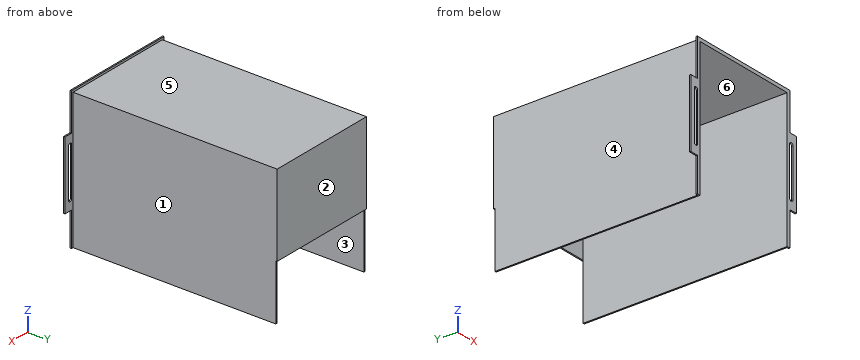
```python
from build123d import *

# Parameters (mm, degrees)
BOSS_EXTRUDE1_DEPTH     = 300
SKETCH4_W               = 15
SKETCH4_H               = 100
BOSS_EXTRUDE3_DEPTH     = 2
CUT_EXTRUDE2_DEPTH      = 402.657814564
CUT_EXTRUDE2_DEPTH_BACK = 402.657814564
SKETCH6_W               = 164
SKETCH6_H               = 120
BOSS_EXTRUDE4_DEPTH     = 2
BOSS_EXTRUDE5_DEPTH     = 2


with BuildPart() as part:
    # Sketch1 → Boss-Extrude1 (new body)
    with BuildSketch(Plane(origin=(0, 0, 0), x_dir=(1, 0, 0), z_dir=(0, 1, 0))):
        Polygon((160, 0), (160, 200), (162, 200), (162, -2), (-2, -2), (-2, 200), (0, 200), (0, 0), align=None)
    extrude(amount=BOSS_EXTRUDE1_DEPTH)

    # Sketch4 → Boss-Extrude3 (add)
    with BuildSketch(Plane.XZ):
        with Locations((-9.5, -100)):
            Rectangle(SKETCH4_W, SKETCH4_H)
        with Locations((169.5, -100)):
            Rectangle(SKETCH4_W, SKETCH4_H)
    extrude(amount=-BOSS_EXTRUDE3_DEPTH)

    # Sketch5 → Cut-Extrude2 (cut, two sides: drawn at the far end of the back side and taken through both)
    with BuildSketch(Plane.XZ.offset(-CUT_EXTRUDE2_DEPTH_BACK)):
        with BuildLine():
            Line((-4.4, -65), (-4.4, -135))
            ThreePointArc((-4.4, -135), (-7.5, -138.1), (-10.6, -135))
            Line((-10.6, -135), (-10.6, -65))
            ThreePointArc((-10.6, -65), (-7.5, -61.9), (-4.4, -65))
        make_face()
        with BuildLine():
            Line((170.6, -65), (170.6, -135))
            ThreePointArc((170.6, -135), (167.5, -138.1), (164.4, -135))
            Line((164.4, -135), (164.4, -65))
            ThreePointArc((164.4, -65), (167.5, -61.9), (170.6, -65))
        make_face()
    extrude(amount=CUT_EXTRUDE2_DEPTH + CUT_EXTRUDE2_DEPTH_BACK, mode=Mode.SUBTRACT)

    # Sketch6 → Boss-Extrude4 (add)
    with BuildSketch(Plane(origin=(0, 300, 0), x_dir=(1, 0, 0), z_dir=(0, 1, 0))):
        with Locations((80, 58)):
            Rectangle(SKETCH6_W, SKETCH6_H)
    extrude(amount=BOSS_EXTRUDE4_DEPTH)

    # Sketch7 → Boss-Extrude5 (add)
    with BuildSketch(Plane.XZ):
        Polygon((-2, -200), (-2, 2), (162, 2), (162, -200), (165, -200), (165, -137.966768061), (163.387303915, -137.966768061), (163.387303915, -56.304675841), (165, -56.304675841), (165, 5), (-5, 5), (-5, -59.253655593), (-3.5, -59.253655593), (-3.5, -137.966768061), (-5, -137.966768061), (-5, -200), align=None)
    extrude(amount=-BOSS_EXTRUDE5_DEPTH)


solid = part.part
```
Here's how the part is built. I have some questions about the finished solid (model axes, mm). Face numbers are marked on the shaded views. A direction names the side the tool comes from. Coordinates: 2 decimals unless noted, no trailing zeros. Order: outer loops, then holes, each group sorted by start corner. A loop starts at its lowest first (then second) coordinate and runs counter-clockwise, first axis right, second up. Notation, with made-up numbers: (67.25, -25.5) -> (111.25, -25.5) arc R20 cw to (111.25, 6.5) -> close; hole circle Ø9 at (3, -29.5). An arc over 180 degrees is marked (long way). Return JSON: item names as keys, results as strings.
1) If I drill on probe 1 along X at (y, z) = (256.5, -40.5); probe 2 along Y at (x, z) = (1.5, -29); probe 3 along Z at (x, y) = (141.5, 109), over which ranges is the centre line in solid material (lowest first)?
Conclusion:
{"probe 1": "x = -2 to 0, 160 to 162", "probe 2": "y = 300 to 302", "probe 3": "z = 0 to 2"}
2) Thinking about a two-plate mould opening in X: for the marked faces 1, 2, 3 and 4, which applies, +X half, -X half, draft (parallel to the pull), parting line (faces both ways), or undercut?
Conclusion:
{"face 1": "+X half", "face 2": "draft", "face 3": "undercut", "face 4": "-X half"}
3) On a 3-axis mill with a long thin cutter (end or side, diameter ignored), from which of +Z, -Z, +X, -X, +Y, -Y can I reach the whole of each face in a straight line? I mean the marked faces 5 and 6. Say none if no direction works.
Conclusion:
{"face 5": "+Z, +X, -X, +Y", "face 6": "-Z, -Y"}
4) I'm going to push flat-ended pins straight in: P1, Ø1, axis at x = 34.5, z = -115.5, coming from the -Y side; P2, Ø6, axis at y = 222, z = -157, coming from the +X side; P3, Ø1, axis at x = 172.5, y = 1.5, coming from the -Z side. Where does each tip first touch, or does it pass through?
Conclusion:
{"P1": "stops at y = 300", "P2": "stops at x = 162", "P3": "stops at z = -150"}
5) If we section it at A-A on z = -125: List the corners of the cut face in (x, y) for me, plus the area to 3 significant figures.
Conclusion:
{"outline": "(-17, 0) -> (-10.6, 0) -> (-10.6, 2) -> (-17, 2) -> close; (-4.4, 0) -> (0, 0) -> (0, 300) -> (-2, 300) -> (-2, 2) -> (-4.4, 2) -> close; (160, 0) -> (164.4, 0) -> (164.4, 2) -> (162, 2) -> (162, 300) -> (160, 300) -> close; (170.6, 0) -> (177, 0) -> (177, 2) -> (170.6, 2) -> close", "area": "1,240 mm²"}
6) If we section it at C-C on z = -81: List the corners of the cut face in (x, y) for me, plus the area to 3 significant figures.
Conclusion:
{"outline": "(-17, 0) -> (-10.6, 0) -> (-10.6, 2) -> (-17, 2) -> close; (-4.4, 0) -> (0, 0) -> (0, 300) -> (160, 300) -> (160, 0) -> (164.4, 0) -> (164.4, 2) -> (162, 2) -> (162, 302) -> (-2, 302) -> (-2, 2) -> (-4.4, 2) -> close; (170.6, 0) -> (177, 0) -> (177, 2) -> (170.6, 2) -> close", "area": "1,560 mm²"}
7) If we section it at B-B on z = -162: List the corners of the cut face in (x, y) for me.
Conclusion:
{"outline": "(-5, 0) -> (0, 0) -> (0, 300) -> (-2, 300) -> (-2, 2) -> (-5, 2) -> close; (160, 0) -> (165, 0) -> (165, 2) -> (162, 2) -> (162, 300) -> (160, 300) -> close"}
8) If we section it at D-D on x = 104: List the corners of the cut face in (y, z) for me, plus the area to 3 significant figures.
Conclusion:
{"outline": "(0, 0) -> (300, 0) -> (300, -118) -> (302, -118) -> (302, 2) -> (2, 2) -> (2, 5) -> (0, 5) -> close", "area": "846 mm²"}
